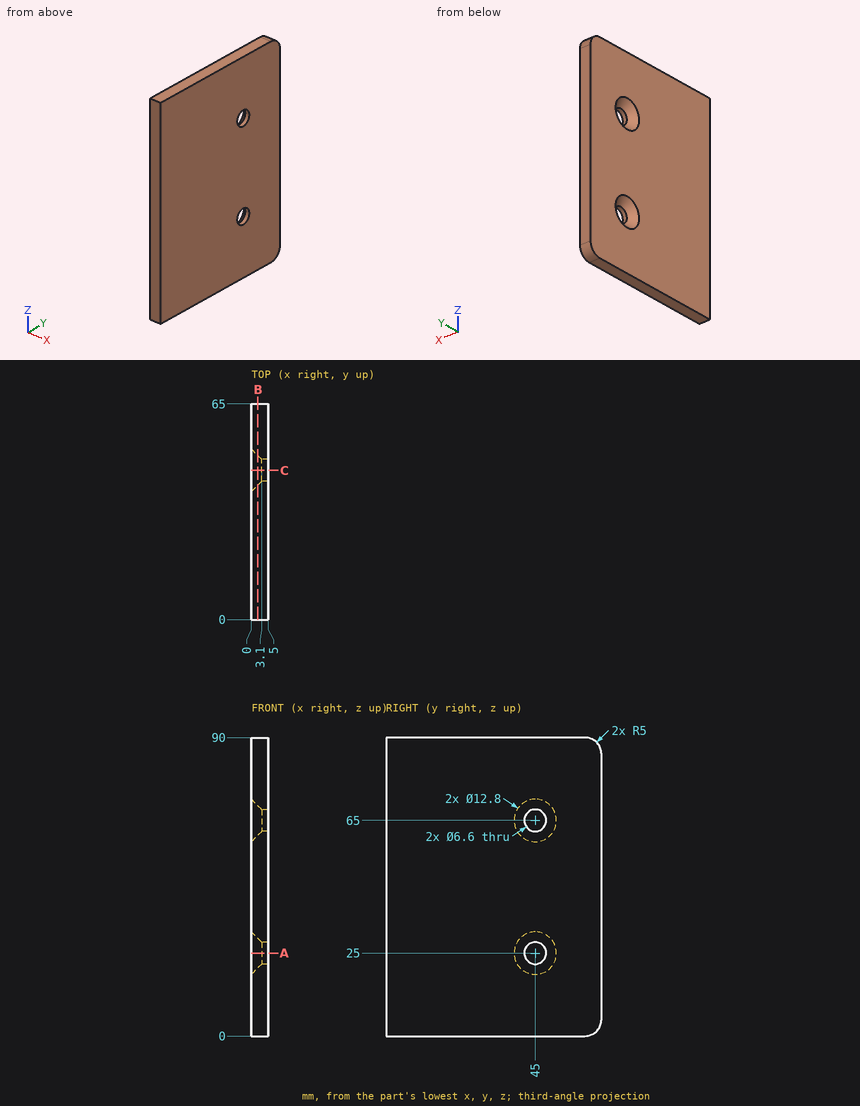
Can you work these out from the drawing? Everything is in mm from the part's minimum corner. Give positions to 0.01 mm unless a question says otherwise; leave off trailing zeros. Write each loop counter-clockwise with the first axis right and the second up, starting at its lowest first coordinate (ties: lowest second). Pieces come first, ordered by that corner, then holes. Notation, with made-up numbers: M 44,50 L 67,50 A7 ccw 67,60 Z; hole C 62,11 d5. An arc over 180 degrees is marked long. Answer in a Markdown table with one row per item. Add a question column.
Item 1: For pin 1 Ø8.5 at (y, z) = (45, 65) entering from -X; pin 2 Ø7.5 at (y, z) = (45, 25) entering from -X, each with a flat end and sliding along its axis, tell me the tip position at first contact or that it passes through.
Item 2: Imagine slicing it at A-A, the plane z = 25. Write out the boundary of the cut face in (x, y).
Item 3: Imagine slicing it at B-B, the plane x = 1.95. Write out the boundary of the cut face in (y, z), plus the area to 3 significant figures.
Item 4: Please list where these lines run through material, in increasing order: L1, parallel to Z at x = 3.8, y = 45; L2, parallel to Y at x = 3.85, z = 25; L3, parallel to Z at x = 1.35, y = 43.5.
Item 5: Imagine slicing it at C-C, the plane y = 45. Write out the boundary of the cut face in (x, z).
Evaluation:
| question | item | result |
|---|---|---|
| 1 | pin 1 | stops at x = 2.15 |
| 1 | pin 2 | stops at x = 2.65 |
| 2 | outline | M 0,0 L 5,0 L 5,41.7 L 3.1,41.7 L 0,38.6 Z; M 0,51.4 L 3.1,48.3 L 5,48.3 L 5,65 L 0,65 Z |
| 3 | outline | M 0,0 L 60,0 A5 ccw 65,5 L 65,85 A5 ccw 60,90 L 0,90 Z; hole C 45,25 d8.9; hole C 45,65 d8.9 |
| 3 | area | 5,710 mm² |
| 4 | L1 | z = 0 to 21.7, 28.3 to 61.7, 68.3 to 90 |
| 4 | L2 | y = 0 to 41.7, 48.3 to 65 |
| 4 | L3 | z = 0 to 20.18, 29.82 to 60.18, 69.82 to 90 |
| 5 | outline | M 0,0 L 5,0 L 5,21.7 L 3.1,21.7 L 0,18.6 Z; M 0,31.4 L 3.1,28.3 L 5,28.3 L 5,61.7 L 3.1,61.7 L 0,58.6 Z; M 0,71.4 L 3.1,68.3 L 5,68.3 L 5,90 L 0,90 Z |
